Can you work these out from the model? Positions are in its coordinate system, mm. Face numbers are marked on the shaded views. A direction names the side the tool comes from. Coordinates: 2 decimals unless noted, no trailing zeros. Return JSON: item names as keys, results as strings. Group by question number.
1) For pin 1 Ø12 at (x, z) = (-441, 11) entering from +Y; pin 2 Ø10 at (x, z) = (-296.5, 22.5) entering from -Y; pin 3 Ø5 at (x, z) = (296.5, -22.5) entering from -Y; pin 4 Ø8.5 at (x, z) = (0, -12.5) entering from +Y, each with a flat end and sliding along its axis, tell me the tip position at first contact or that it passes through.
2) Which directions (+Z, -Z, +X, -X, +Y, -Y) give clear straight access to the entire face, cutting with the end or side of a thin tool? Please do the marked faces 1 and 2.
3) If we mould it in two halves opening along X, with no side actions, what happens to the marked faces 3 and 4? For each: pulls with the +X half, pulls with the -X half, needs draft (parallel to the pull), parting line crosses it, or undercut.
4) Imagine slicing it at A-A (y = 12.75). Give the number of separate pieces and of enclosed holes in the cut face, and give its area (3 significant figures).
5) If I drill on line 1 along Z through (x, y) = (353.5, 9.75); line 2 along Z through (x, y) = (440, 11.5); line 3 along X through (y, z) = (6.5, -26), over which ranges is the centre line in solid material (lowest first)?
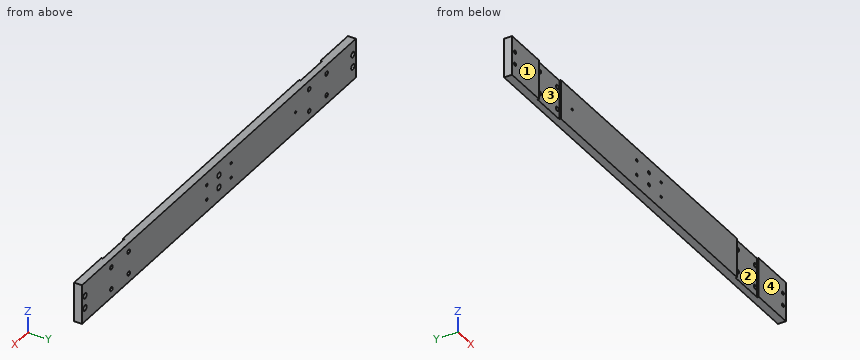
```python
from build123d import *

# Parameters (mm, degrees)
SKETCH_1_W                = 900
SKETCH_1_H                = 80
EXTRUDE_1_DEPTH           = 16
SKETCH_2_W                = 71.098057304
SKETCH_2_H                = 80
CUT_EXTRUDE_1_DEPTH       = 3
HOLE_WIZARD_8_5_8_5_1_D   = 8.5
HOLE_WIZARD_M6_1_D        = 5
HOLE_WIZARD_1_D           = 6.6
HOLE_WIZARD_1_CBORE_D     = 11
HOLE_WIZARD_1_CBORE_DEPTH = 6.8
PATTERN_LINEAR_1_COUNT    = 3
PATTERN_LINEAR_1_PITCH    = 440
HOLE_WIZARD_M5_1_D        = 4.2


with BuildPart() as part:
    # 草图1 → 凸台-拉伸1 (new body)
    with BuildSketch(Plane(origin=(0, 0, 0), x_dir=(1, 0, 0), z_dir=(0, 1, 0))):
        Rectangle(SKETCH_1_W, SKETCH_1_H)
    extrude(amount=EXTRUDE_1_DEPTH)

    # 草图2 → 切除-拉伸1 (cut)
    with BuildSketch(Plane.XZ):
        with Locations((-325, 0)):
            Rectangle(SKETCH_2_W, SKETCH_2_H)
        with Locations((325, 0)):
            Rectangle(SKETCH_2_W, SKETCH_2_H)
    extrude(amount=-CUT_EXTRUDE_1_DEPTH, mode=Mode.SUBTRACT)

    # Ø8.5 (8.5) 直径孔1 (through all)
    with Locations(Plane(origin=(0, 16, 0), x_dir=(1, 0, 0), z_dir=(0, 1, 0))):
        with Locations((-353.5, 22.5), (-296.5, 22.5), (-353.5, -22.5), (-296.5, -22.5)):
            hole_wizard_8_5_8_5_1 = Hole(HOLE_WIZARD_8_5_8_5_1_D / 2)

    # 镜向1: Ø8.5 (8.5) 直径孔1 across plane
    add(hole_wizard_8_5_8_5_1.mirror(Plane(origin=(0, 0, 0), x_dir=(0, 0, 1), z_dir=(1, 0, 0))), mode=Mode.SUBTRACT)

    # M6 螺纹孔1 (through all)
    with Locations(Plane(origin=(0, 16, 0), x_dir=(1, 0, 0), z_dir=(0, 1, 0))):
        with Locations((-40, 15), (40, 15), (-40, -15), (40, -15)):
            Hole(HOLE_WIZARD_M6_1_D / 2)

    # 打孔尺寸(%根据)内六角圆柱头螺钉的类型1 (through all)
    with Locations(Plane(origin=(0, 16, 0), x_dir=(1, 0, 0), z_dir=(0, 1, 0))):
        with Locations((-440, 12.5), (-440, -12.5)):
            hole_wizard_1 = CounterBoreHole(HOLE_WIZARD_1_D / 2, HOLE_WIZARD_1_CBORE_D / 2, HOLE_WIZARD_1_CBORE_DEPTH)

    # 阵列(线性)1: 打孔尺寸(%根据)内六角圆柱头螺钉的类型1 ×3
    with Locations(*[(i * PATTERN_LINEAR_1_PITCH, 0, 0) for i in range(1, PATTERN_LINEAR_1_COUNT)]):
        add(hole_wizard_1, mode=Mode.SUBTRACT)

    # M5 螺纹孔1 (through all)
    with Locations(Plane(origin=(0, 16, 0), x_dir=(1, 0, 0), z_dir=(0, 1, 0))):
        with Locations((-252, 0)):
            Hole(HOLE_WIZARD_M5_1_D / 2)


solid = part.part
```
Calculated:
{
 "1": {"pin 1": "y = 16", "pin 2": "y = 3", "pin 3": "through", "pin 4": "y = 9.2"},
 "2": {"face 1": "+Z, -Z, +X, -X, -Y", "face 2": "+Z, -Z, -Y"},
 "3": {"face 3": "undercut", "face 4": "needs draft"},
 "4": {"separate pieces": "1", "enclosed holes": "19", "area": "70,900 mm2"},
 "5": {"line 1": "-40 to -26.75, -18.25 to 18.25, 26.75 to 40", "line 2": "-40 to -18, -7 to 7, 18 to 40", "line 3": "-450 to -355.91, -351.09 to -298.91, -294.09 to 294.09, 298.91 to 351.09, 355.91 to 450"}
}
